```python
from build123d import *

# Parameters (mm, degrees)
SKETCH1_R           = 40
SKETCH1_R_2         = 27.5
BOSS_EXTRUDE1_DEPTH = 25


with BuildPart() as part:
    # Sketch1 → Boss-Extrude1 (new body)
    with BuildSketch(Plane.XY):
        with BuildLine():
            Line((-175.1, -115), (175.1, -115))
            Line((175.1, -115), (175.1, -80))
            Line((175.1, -80), (205.1, -80))
            Line((205.1, -80), (130.002057063, -4.902057063))
            ThreePointArc((130.002057063, -4.902057063), (106.058771733, 22.112599839), (85.533522855, 51.807494323))
            ThreePointArc((85.533522855, 51.807494323), (-8.510447338, 99.637203323), (-93.080630623, 36.551281821))
            ThreePointArc((-93.080630623, 36.551281821), (-164.286464639, -24.475575679), (-254.730193824, 0.313131132))
            ThreePointArc((-254.730193824, 0.313131132), (-344.272458908, -0.069434909), (-348.468561101, -89.514145872))
            ThreePointArc((-348.468561101, -89.514145872), (-276.775086195, -205.471406239), (-244.984042874, -338.043538078))
            ThreePointArc((-244.984042874, -338.043538078), (-232.286931391, -364.340599202), (-205.1, -375))
            Line((-205.1, -375), (-205.1, -80))
            Line((-205.1, -80), (-175.1, -80))
            Line((-175.1, -80), (-175.1, -115))
        make_face()
        Circle(SKETCH1_R, mode=Mode.SUBTRACT)
        with Locations((-299.3, -47)):
            Circle(SKETCH1_R_2, mode=Mode.SUBTRACT)
    extrude(amount=BOSS_EXTRUDE1_DEPTH)


solid = part.part
```
Source: CAD feature listing. Evaluate the final solid. Frame: model axes, mm. A direction names the side the tool comes from. Round coordinates to 2 decimals unless told otherwise and drop trailing zeros. Loops run counter-clockwise (first coordinate to the right, second up) from the corner with the lowest first, then second, coordinate; pieces in that order, holes last. Notation, with made-up numbers: M 42,50.5 L 72,50.5 A18 ccw 72,78.5 Z; hole C -8.75,85.25 d6. An arc over 180 degrees is marked long. Use a Markdown table: item, result. Add a question column.
1. Cut plane C-C, the plane z = 17. Output: boundary loops of the cut face in (x, y), and give its area (3 significant figures).
2. Pull-direction query (Y, two-part tool) for faces 4 (the cylindrical face through (-8.67, -39.05, 12.32)), 5 (the cylindrical face through (-277.516, -203.704, 12.325)), 6 (the flat face through (-175.1, -97, 12)); classes: +Y half, -Y half, draft (parallel to the pull), parting line (faces both ways), or undercut.
3. Cut plane B-B, the plane y = -47. Output: boundary loops of the cut face in (x, z), and give its area (3 significant figures).
4. Contact query for flat-ended pins moving along their axis: pin 1 (1.5 mm diameter, centred on y = -34.5, z = 16, fed in from -X); pin 2 (3 mm diameter, centred on x = -202.5, z = 22, fed in from -Y); pin 3 (12 mm diameter, centred on y = -283.5, z = 14.5, fed in from -X). Output: stop coordinate, or through.
5. Set-up query: faces 1 (the flat face through (-190, -80, 12)), 2 (the flat face through (-123, -84, 25)), 3 (the flat face through (190, -80, 12)). Return all of +Z, -Z, +X, -X, +Y, -Y with unobstructed straight access to the full face (end or side cutting, diameter ignored); none if empty.
6. Cut plane A-A, the plane x = 0. Output: boundary loops of the cut face in (y, z).
7. Cut plane D-D, the plane y = 59.5. Output: boundary loops of the cut face in (x, z), and give its area (3 significant figures).
8. Ray query, line 1 along Y through (x, z) = (0, 15.25); line 2 along X through (y, z) = (-32.5, 19.25); line 3 along X through (y, z) = (-17.5, 22). Return the intervals inside material, ascending. Write a range as [from, to].
Solution:
| question | item | result |
|---|---|---|
| 1 | outline | M -348.47,-89.51 A430 cw -244.98,-338.04 A40 ccw -205.1,-375 L -205.1,-80 L -175.1,-80 L -175.1,-115 L 175.1,-115 L 175.1,-80 L 205.1,-80 L 130,-4.9 A300 cw 85.53,51.81 A100 ccw -93.08,36.55 A100 cw -254.73,0.31 A65 ccw Z; hole C -299.3,-47 d55; hole C 0,0 d80 |
| 1 | area | 83,200 mm2 |
| 2 | face 4 | undercut |
| 2 | face 5 | -Y half |
| 2 | face 6 | draft |
| 3 | outline | M -364.3,0 L -326.8,0 L -326.8,25 L -364.3,25 Z; M -271.8,0 L 172.1,0 L 172.1,25 L -271.8,25 Z |
| 3 | area | 12,000 mm2 |
| 4 | pin 1 | stops at x = -363.23 |
| 4 | pin 2 | stops at y = -80 |
| 4 | pin 3 | stops at x = -253.97 |
| 5 | face 1 | +Z, -Z, -Y |
| 5 | face 2 | +Z, +X, -X, +Y, -Y |
| 5 | face 3 | +Z, -Z, +X, -Y |
| 6 | outline | M -115,0 L -40,0 L -40,25 L -115,25 Z; M 40,0 L 100,0 L 100,25 L 40,25 Z |
| 7 | outline | M -80.37,0 L 80.37,0 L 80.37,25 L -80.37,25 Z |
| 7 | area | 4,020 mm2 |
| 8 | line 1 | y = [-115, -40], [40, 100] |
| 8 | line 2 | x = [-362.66, -322.67], [-275.93, -23.32], [23.32, 157.6] |
| 8 | line 3 | x = [-357.22, -228.48], [-143.84, -35.97], [35.97, 142.6] |
